from build123d import *

# Parameters (mm, degrees)
EXTRUDE_THIN1_DEPTH      = 15
EXTRUDE_THIN1_DEPTH_BACK = 15
SKETCH2_R                = 12.5
CUT_EXTRUDE1_DEPTH       = 52
CUT_EXTRUDE2_DEPTH       = 52


with BuildPart() as part:
    # Sketch1 → Extrude-Thin1 (new, two sides: drawn at the far end of the back side and taken through both)
    with BuildSketch(Plane(origin=(-52.015152818, 0, 189.77373053), x_dir=(0.9644293353148398, 0, 0.2643407974266862), z_dir=(-0.2643407974266862, 0, 0.9644293353148398)).offset(-EXTRUDE_THIN1_DEPTH_BACK)):
        Polygon((-6.089055059, 159.279680039), (25.645783745, 151.090927797), (451.524648913, 41.198562071), (462.768022338, 84.771335153), (36.889157171, 194.663700878), (5.154318366, 202.85245312), align=None)
    extrude(amount=EXTRUDE_THIN1_DEPTH + EXTRUDE_THIN1_DEPTH_BACK)

    # Sketch2 → Cut-Extrude1 (cut)
    with BuildSketch(Plane(origin=(-55.98026478, 0, 204.240170559), x_dir=(0.9644293353148398, 0, 0.26434079742668615), z_dir=(-0.26434079742668615, 0, 0.9644293353148398))):
        with Locations((432.939239469, 69.231267182)):
            Circle(SKETCH2_R)
        with Locations((384.525047156, 81.723904321)):
            Circle(SKETCH2_R)
        with Locations((336.110854844, 94.216541461)):
            Circle(SKETCH2_R)
        with Locations((287.696662531, 106.7091786)):
            Circle(SKETCH2_R)
        with Locations((239.282470218, 119.20181574)):
            Circle(SKETCH2_R)
        with Locations((190.868277905, 131.694452879)):
            Circle(SKETCH2_R)
        with Locations((142.454085592, 144.187090019)):
            Circle(SKETCH2_R)
        with Locations((94.03989328, 156.679727158)):
            Circle(SKETCH2_R)
        with Locations((45.625700967, 169.172364298)):
            Circle(SKETCH2_R)
    extrude(amount=-CUT_EXTRUDE1_DEPTH, mode=Mode.SUBTRACT)

    # Sketch3 → Cut-Extrude2 (cut)
    with BuildSketch(Plane(origin=(47.64042684, 191.43608201, 13.057782421), x_dir=(0.9705337279727567, -0.24040671124001461, -0.01639805043483442), z_dir=(0.24096531465607895, 0.9682838462558588, 0.06604627326849857))):
        Polygon((359.082690346, -298.87451483), (355.26956046, -312.345225296), (-91.768329186, -185.803010492), (-87.955199299, -172.332300026), align=None)
    extrude(amount=-CUT_EXTRUDE2_DEPTH, mode=Mode.SUBTRACT)


solid = part.part
Can you work these out from the model? Positions are in its coordinate system, mm. A direction names the side the tool comes from. Round coordinates to 2 decimals unless told otherwise and drop trailing zeros. Write each loop counter-clockwise with the first axis right and the second up, starting at its lowest first coordinate (ties: lowest second). Pieces come first, ordered by that corner, then holes. Notation, with made-up numbers: M 57.5,-14 L 112.5,-14 A19 ccw 112.5,2 Z; hole C -14.75,83.25 d1. An arc over 180 degrees is marked long. Use a Markdown table: item, result.
Item 1: For pin 1 Ø5 at (x, z) = (224.5, 277.5) entering from -Y; pin 2 Ø1 at (x, y) = (10.5, 146) entering from -Z, each with a flat end and sliding along its axis, tell me the tip position at first contact or that it passes through.
Found:
| item | result |
|---|---|
| pin 1 | stops at y = 82.27 |
| pin 2 | stops at z = 191.22 |
Item 2: I want a section at C-C (y = 126). List the corners of the cut face in (x, z) for me, and give its area (3 significant figures).
Found:
| item | result |
|---|---|
| outline | M 62.53,236.72 L 64.65,229.01 L 119.48,244.04 L 117.37,251.75 Z; M 68.35,215.51 L 70.46,207.79 L 125.3,222.82 L 123.18,230.54 Z; M 138.83,257.64 L 140.95,249.92 L 166.79,257 L 164.67,264.72 Z; M 144.65,236.42 L 146.76,228.7 L 172.6,235.79 L 170.49,243.5 Z; M 184.91,270.27 L 187.02,262.55 L 238.35,276.62 L 236.23,284.33 Z; M 190.72,249.05 L 192.84,241.33 L 244.16,255.4 L 242.05,263.12 Z |
| area | 2,190 mm2 |
Item 3: We'd pull the mould along X, two halves only. Please class faces 3 (the face through (280.716, 97.971, 292.436)), 4 (the face through (385.9, 62.68, 321.15)), 5 (the face through (163.18, 128.39, 264.31)): released by +X, released by -X, zero draft, split by the parting line, or undercut.
Found:
| item | result |
|---|---|
| face 3 | undercut |
| face 4 | released by +X |
| face 5 | released by -X |
Item 4: If I drill on line 1 along Z through (x, y) = (158.5, 122); line 2 along Z through (x, y) = (240, 90.5); line 3 along Y through (x, z) = (149.5, 229.5), over which ranges is the centre line in solid material (lowest first)? Write a range as [from, to].
Found:
| item | result |
|---|---|
| line 1 | z = [231.92, 240.22], [254.73, 263.03] |
| line 2 | z = [254.26, 262.55], [277.07, 285.37] |
| line 3 | y = [104.85, 151.32] |
Item 5: I want a section at D-D (x = 34.5). State how many separate pieces and enclosed holes the cut face has, and give its area (3 significant figures).
Found:
| item | result |
|---|---|
| separate pieces | 4 |
| enclosed holes | 0 |
| area | 398 mm2 |
Item 6: I want a section at B-B (x = 153.5). List the corners of the cut face in (y, z) for me.
Found:
| item | result |
|---|---|
| outline | M 101.66,261.66 L 102.23,253.36 L 148.7,253.36 L 148.14,261.66 Z; M 103.22,238.85 L 103.78,230.55 L 150.26,230.55 L 149.69,238.85 Z |
Item 7: I want a section at A-A (y = 100). List the corners of the cut face in (x, z) for me, and give its area (3 significant figures).
Found:
| item | result |
|---|---|
| outline | M 159.71,263.36 L 161.82,255.64 L 213.43,269.79 L 211.31,277.5 Z; M 165.52,242.14 L 167.64,234.43 L 219.24,248.57 L 217.13,256.28 Z; M 231.65,283.08 L 233.77,275.36 L 259.6,282.44 L 257.49,290.16 Z; M 237.47,261.86 L 239.58,254.15 L 265.42,261.23 L 263.3,268.94 Z; M 278.86,296.02 L 280.98,288.3 L 335.52,303.25 L 333.41,310.97 Z; M 284.68,274.8 L 286.79,267.08 L 341.34,282.04 L 339.22,289.75 Z |
| area | 2,190 mm2 |
Item 8: Which directions (+Z, -Z, +X, -X, +Y, -Y) give clear straight access to the entire face, cutting with the end or side of a thin tool? Please do faces 1 (the face through (-44.945, 179.372, 191.813)), 2 (the face through (-7.73, 156.97, 190.56)).
Found:
| item | result |
|---|---|
| face 1 | -Y |
| face 2 | none |
